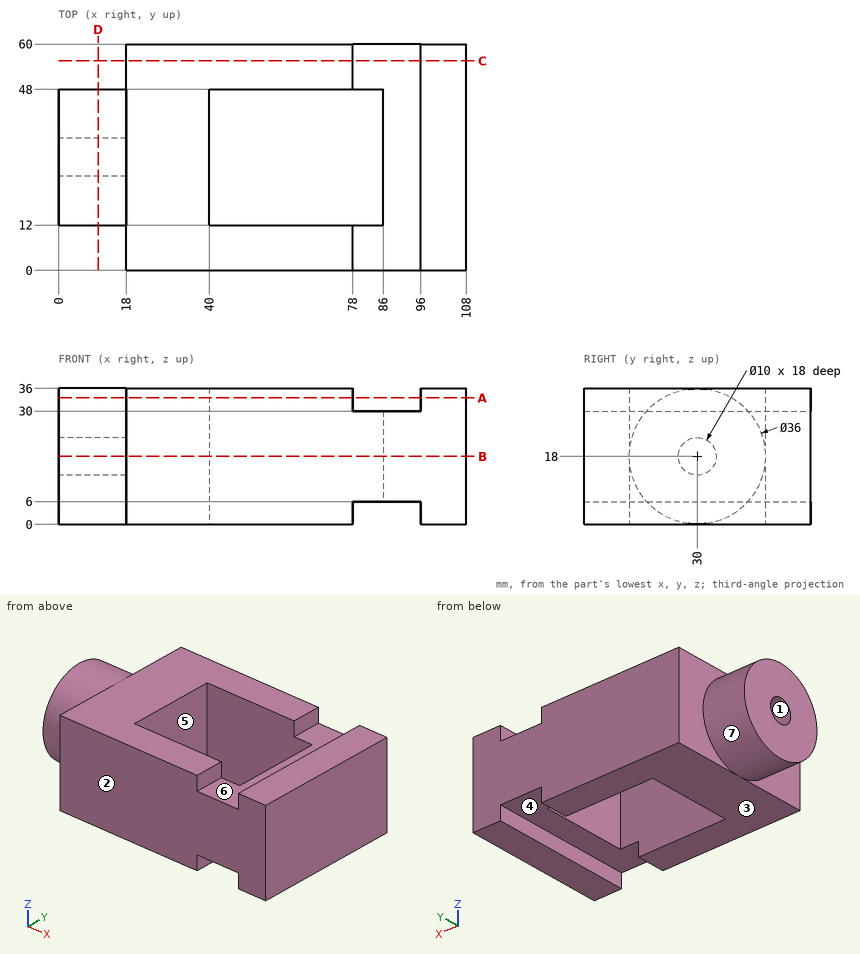
Print and shaded views of the part. All mm, measured from the part's lowest x, y and z. A direction names the side the tool comes from. Round coordinates to 2 decimals unless told otherwise and drop trailing zeros. Write each loop counter-clockwise with the first axis right and the second up, starting at its lowest first coordinate (ties: lowest second). Pieces come first, ordered by that corner, then holes. Notation, with made-up numbers: (29.5, 6.5) -> (80.5, 6.5) arc R21 ccw to (80.5, 23.5) -> close; hole circle Ø8 at (66.25, -23). An arc over 180 degrees is marked (long way). Answer in a Markdown table with one row per item. Add a question column.
Item 1: Mould opens along Y. For the marked faces 1, 2 and 3 say: pulls with the +Y half, pulls with the -Y half, needs draft (parallel to the pull), parting line crosses it, or undercut.
Item 2: Saw through at A-A, the plane z = 33.5. Write the cut outline in (x, y), then the cut area to 3 significant figures.
Item 3: Saw through at D-D, the plane x = 10.5. Write the cut outline in (y, z), then the cut area to 3 significant figures.
Item 4: Saw through at B-B, the plane z = 18. Write the cut outline in (x, y).
Item 5: Saw through at C-C, the plane y = 55.5. Write the cut outline in (x, z), then the cut area to 3 significant figures.
Item 6: Drill centre lines: line 1 (Y direction, x = 74, z = 20); line 2 (X direction, y = 54, z = 32.5); line 3 (Y direction, x = 12, z = 18). Where is each one in solid material? Low to high. Write a range as from..to.
Item 7: Drop flat-ended pins along their axis: pin 1 Ø3 at (y, z) = (16, 4) entering from -X; pin 2 Ø9 at (x, y) = (82.5, 23.5) entering from -Z; pin 3 Ø9 at (x, y) = (86, 19) entering from +Z. Give the stop position or say it passes through.
Item 8: Which spindle directions (+Z, -Z, +X, -X, +Y, -Y) get a long thin tool onto all of the face, cutting with end or side? Do the marked faces 4, 5, 6 and 7. Say none if no direction does.
Findings below:
| question | item | result |
|---|---|---|
| 1 | face 1 | undercut |
| 1 | face 2 | pulls with the -Y half |
| 1 | face 3 | needs draft |
| 2 | outline | (0, 20.85) -> (18, 20.85) -> (18, 0) -> (78, 0) -> (78, 12) -> (40, 12) -> (40, 48) -> (78, 48) -> (78, 60) -> (18, 60) -> (18, 39.15) -> (0, 39.15) -> close; (96, 0) -> (108, 0) -> (108, 60) -> (96, 60) -> close |
| 2 | area | 3,280 mm^2 |
| 3 | outline | circle Ø36 at (30, 18); hole circle Ø10 at (30, 18) |
| 3 | area | 939 mm^2 |
| 4 | outline | (0, 12) -> (18, 12) -> (18, 0) -> (108, 0) -> (108, 60) -> (18, 60) -> (18, 48) -> (0, 48) -> (0, 35) -> (18, 35) -> (18, 25) -> (0, 25) -> close; hole (40, 12) -> (86, 12) -> (86, 48) -> (40, 48) -> close |
| 5 | outline | (18, 0) -> (78, 0) -> (78, 6) -> (96, 6) -> (96, 0) -> (108, 0) -> (108, 36) -> (96, 36) -> (96, 30) -> (78, 30) -> (78, 36) -> (18, 36) -> close |
| 5 | area | 3,020 mm^2 |
| 6 | line 1 | y = 0..12, 48..60 |
| 6 | line 2 | x = 18..78, 96..108 |
| 6 | line 3 | y = 12..25, 35..48 |
| 7 | pin 1 | stops at x = 18 |
| 7 | pin 2 | stops at z = 6 |
| 7 | pin 3 | stops at z = 30 |
| 8 | face 4 | -Z, +Y, -Y |
| 8 | face 5 | +Z, -Z |
| 8 | face 6 | +Z, +Y, -Y |
| 8 | face 7 | -X |
